Check sheet for the modelled part. Datum: model origin and axes. Units: mm. Face numbers are marked on the shaded views. Give positions to 0.01 mm unless a question says otherwise; leave off trailing zeros. Write each loop counter-clockwise with the first axis right and the second up, starting at its lowest first coordinate (ties: lowest second). Pieces come first, ordered by that corner, then holes. Notation, with made-up numbers: (7, 11.25) -> (26, 11.25) arc R29 cw to (26, 49.25) -> close; hole circle Ø5 at (42, 71). An arc over 180 degrees is marked (long way). Answer as a JSON object with one key per item and string values.
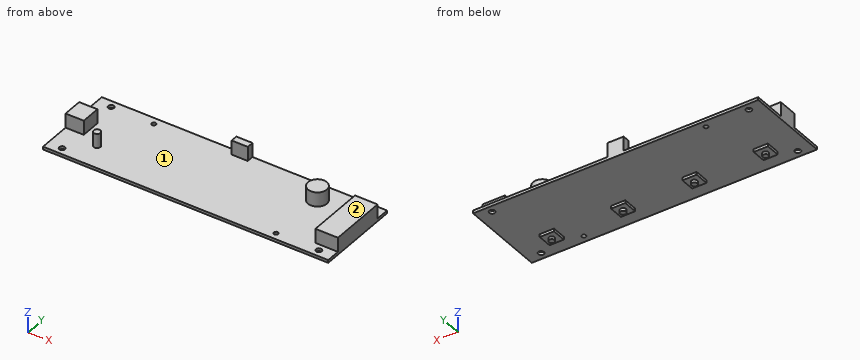
from build123d import *

# Parameters (mm, degrees)
SKETCH1_W           = 100
SKETCH1_H           = 30
SKETCH1_R           = 1
BOSS_EXTRUDE1_DEPTH = 1
SKETCH2_R           = 3.312148645
SKETCH2_R_2         = 1.182707094
SKETCH2_W           = 7.897065894
SKETCH2_H           = 20.201539664
SKETCH2_W_2         = 5.658967966
SKETCH2_H_2         = 2.382698796
SKETCH2_W_3         = 6.371052581
SKETCH2_H_3         = 6.939357654
BOSS_EXTRUDE2_DEPTH = 5
SKETCH3_W           = 5
SKETCH3_H           = 5
BOSS_EXTRUDE3_DEPTH = 1
SKETCH4_R           = 1
BOSS_EXTRUDE4_DEPTH = 1
SKETCH5_R           = 0.75
CUT_EXTRUDE1_DEPTH  = 10


with BuildPart() as part:
    # Sketch1 → Boss-Extrude1 (new body)
    with BuildSketch(Plane.XY):
        Rectangle(SKETCH1_W, SKETCH1_H)
        with Locations((-45, -12.5)):
            Circle(SKETCH1_R, mode=Mode.SUBTRACT)
        with Locations((-45, 12.5)):
            Circle(SKETCH1_R, mode=Mode.SUBTRACT)
        with Locations((45, 12.5)):
            Circle(SKETCH1_R, mode=Mode.SUBTRACT)
        with Locations((45, -12.5)):
            Circle(SKETCH1_R, mode=Mode.SUBTRACT)
    extrude(amount=BOSS_EXTRUDE1_DEPTH)

    # Sketch2 → Boss-Extrude2 (add)
    with BuildSketch(Plane.XY.offset(1)):
        with Locations((30.440398969, 7.974336126)):
            Circle(SKETCH2_R)
        with Locations((-37.372165455, -5.749563916)):
            Circle(SKETCH2_R_2)
        with Locations((46.051467053, 0.07257894)):
            Rectangle(SKETCH2_W, SKETCH2_H)
        with Locations((0, 13.808650602)):
            Rectangle(SKETCH2_W_2, SKETCH2_H_2)
        with Locations((-46.814473709, 0)):
            Rectangle(SKETCH2_W_3, SKETCH2_H_3)
    extrude(amount=BOSS_EXTRUDE2_DEPTH)

    # Sketch3 → Boss-Extrude3 (add)
    with BuildSketch(Plane(origin=(0, 0, 0), x_dir=(-1, 0, 0), z_dir=(0, 0, -1))):
        with Locations((-12.5, -7)):
            Rectangle(SKETCH3_W, SKETCH3_H)
        with Locations((-37.5, -7)):
            Rectangle(SKETCH3_W, SKETCH3_H)
        with Locations((37.5, -7)):
            Rectangle(SKETCH3_W, SKETCH3_H)
        with Locations((12.5, -7)):
            Rectangle(SKETCH3_W, SKETCH3_H)
    extrude(amount=BOSS_EXTRUDE3_DEPTH)

    # Sketch4 → Boss-Extrude4 (add)
    with BuildSketch(Plane(origin=(0, 0, -1), x_dir=(-1, 0, 0), z_dir=(0, 0, -1))):
        with Locations((-37.5, -7)):
            Circle(SKETCH4_R)
        with Locations((-12.5, -7)):
            Circle(SKETCH4_R)
        with Locations((12.5, -7)):
            Circle(SKETCH4_R)
        with Locations((37.5, -7)):
            Circle(SKETCH4_R)
    extrude(amount=BOSS_EXTRUDE4_DEPTH)

    # Sketch5 → Cut-Extrude1 (cut)
    with BuildSketch(Plane.XY.offset(1)):
        with Locations((30, -12.5)):
            Circle(SKETCH5_R)
        with Locations((-30, 12.5)):
            Circle(SKETCH5_R)
    extrude(amount=-CUT_EXTRUDE1_DEPTH, mode=Mode.SUBTRACT)


solid = part.part
1. Sectioned sample at C-C, the plane x = -37.5. Enter the section's corners in (y, z), plus the area to 3 significant figures.
Determined:
{"outline": "(-15, 0) -> (-9.5, 0) -> (-9.5, -1) -> (-8, -1) -> (-8, -2) -> (-6, -2) -> (-6, -1) -> (-4.5, -1) -> (-4.5, 0) -> (15, 0) -> (15, 1) -> (-4.57, 1) -> (-4.57, 6) -> (-6.93, 6) -> (-6.93, 1) -> (-15, 1) -> close", "area": "48.8 mm^2"}
2. Go/stop test with flat-tipped pins: P1, Ø1.5, axis at x = -1, z = 4, coming from the -Y side; P2, Ø12, axis at x = -28, y = -11, coming from the -Z side; P3, Ø3, axis at y = -7, z = 4.5, coming from the -X side; P4, Ø1.8, axis at x = -45, y = 12.5, coming from the -Z side. Record where each tip stops, or that it passes through.
Determined:
{"P1": "y = 12.62", "P2": "z = 0", "P3": "x = -38.55", "P4": "through"}
3. Sectioned sample at B-B, the plane z = 3.25. Enter the section's corners in (x, y).
Determined:
{"outline": "(-50, -3.47) -> (-43.63, -3.47) -> (-43.63, 3.47) -> (-50, 3.47) -> close; circle Ø2.37 at (-37.37, -5.75); (-2.83, 12.62) -> (2.83, 12.62) -> (2.83, 15) -> (-2.83, 15) -> close; circle Ø6.62 at (30.44, 7.97); (42.1, -10.03) -> (50, -10.03) -> (50, 10.17) -> (42.1, 10.17) -> close"}
4. Sectioned sample at A-A, the plane x = -12.5. Enter the section's corners in (y, z).
Determined:
{"outline": "(-15, 0) -> (-9.5, 0) -> (-9.5, -1) -> (-8, -1) -> (-8, -2) -> (-6, -2) -> (-6, -1) -> (-4.5, -1) -> (-4.5, 0) -> (15, 0) -> (15, 1) -> (-15, 1) -> close"}
5. Scan lines: L1, parallel to Y at x = 45, z = 0.7; L2, parallel to Y at x = -30, z = 0.2; L3, parallel to X at y = 2, z = 3.5. Record each from-to range of solid material in increasing order. Write a range as [from, to].
Determined:
{"L1": "[-15, -13.5], [-11.5, 11.5], [13.5, 15]", "L2": "[-15, 11.75], [13.25, 15]", "L3": "[-50, -43.63], [42.1, 50]"}
6. Sectioned sample at D-D, the plane x = 28. Enter the section's corners in (y, z), plus the area to 3 significant figures.
Determined:
{"outline": "(-15, 0) -> (15, 0) -> (15, 1) -> (10.21, 1) -> (10.21, 6) -> (5.73, 6) -> (5.73, 1) -> (-15, 1) -> close", "area": "52.4 mm^2"}
7. Mould release check, pull along X, two halves, no side actions. Record for the marked faces 1 and 2: released by +X, released by -X, zero draft, split by the parting line, or undercut.
Determined:
{"face 1": "undercut", "face 2": "zero draft"}
